Verification items for this drawing (mm, ordinates from the low corner). A direction names the side the tool comes from. Round coordinates to 2 decimals unless told otherwise and drop trailing zeros. Loops run counter-clockwise (first coordinate to the right, second up) from the corner with the lowest first, then second, coordinate; pieces in that order, holes last. Notation, with made-up numbers: M 1.5,-20 L 54.5,-20 A13 cw 54.5,-8 Z; hole C 85.25,4 d9. An arc over 180 degrees is marked long. Write item = value, one per line.
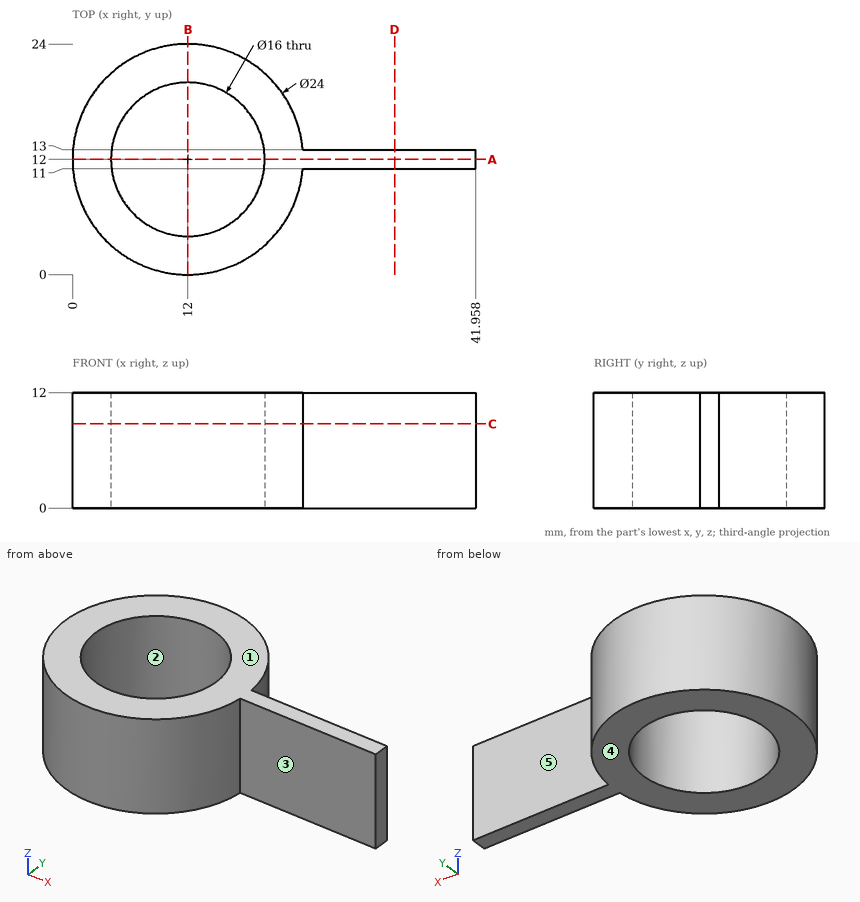
(1) Sectioned sample at B-B on x = 12. Record the cut outline in (y, z).
Result set:
outline = M 0,0 L 4,0 L 4,12 L 0,12 Z; M 20,0 L 24,0 L 24,12 L 20,12 Z
(2) Sectioned sample at A-A on y = 12. Record the cut outline in (x, z).
Result set:
outline = M 0,0 L 4,0 L 4,12 L 0,12 Z; M 20,0 L 41.96,0 L 41.96,12 L 20,12 Z
(3) Tool access check on the marked faces 4 and 5. Record the directions out of +Z, -Z, +X, -X, +Y, -Y that give a thin tool (end or side, any length) a straight path to the whole face; none if there is none.
Result set:
face_4 = -Z, +X, -X, +Y, -Y
face_5 = +Z, -Z, +X, +Y
(4) Sectioned sample at D-D on x = 33.5. Record the cut outline in (y, z), then the cut area to 3 significant figures.
Result set:
outline = M 11,0 L 13,0 L 13,12 L 11,12 Z
area = 24.0 mm2
(5) Material ranges on line 1 along Y through (x, z) = (12, 7.25); line 2 along X through (y, z) = (12.25, 11.25); line 3 along Y through (x, z) = (35.5, 5.75), recorded low to high. Write a range as from..to.
Result set:
line_1 = 0..4, 20..24
line_2 = 0..4, 20..41.96
line_3 = 11..13
(6) Depth check by flat-ended pin: pin 1 Ø4 at (x, z) = (24.5, 6.5) entering from -Y; pin 2 Ø1 at (x, z) = (17.5, 2) entering from +Y; pin 3 Ø3.5 at (x, z) = (29, 6) entering from +Y. Enter the tip coordinate at first touch or a pass-through.
Result set:
pin_1 = 6.19
pin_2 = 22.91
pin_3 = 13
(7) Release check for a two-part mould opening along Y. For the marked faces 1, 2 and 3 record: released by +Y, released by -Y, zero draft, split by the parting line, or undercut.
Result set:
face_1 = zero draft
face_2 = undercut
face_3 = released by -Y
(8) Sectioned sample at C-C on z = 8.75. Record the cut outline in (x, y).
Result set:
outline = M 23.96,11 L 41.96,11 L 41.96,13 L 23.96,13 A12 ccw long Z; hole C 12,12 d16
